Could you check a few things on this model? Use its own coordinates, in mm. A direction names the side the tool comes from. Give positions to 0.01 mm unless a question says otherwise; leave off trailing zeros. Write each loop counter-clockwise with the first axis right and the second up, starting at its lowest first coordinate (ties: lowest second). Pieces come first, ordered by that corner, then holes. Notation, with made-up numbers: (-39, -34.5) -> (-24, -34.5) arc R22 ccw to (-24, -13.5) -> close; hole circle Ø4 at (17, -36). An arc over 180 degrees is marked (long way). Write item = value, one per line. Start each with the question number.
```python
from build123d import *

# Parameters (mm, degrees)
BASE_BLOCK_DEPTH             = 80
UPRIGHT_NOTCHES_SKETCH_W     = 20
UPRIGHT_NOTCHES_SKETCH_H     = 10
UPRIGHT_TOP_NOTCHES_DEPTH    = 15
SADDLE_BORE_SKETCH_R         = 25
SADDLE_BORE_50_DEPTH         = 103.46950766
FRONT_SLOPE_CUT_DEPTH        = 111.742945599
FRONT_SLOT_SKETCH_W          = 5
FRONT_SLOT_SKETCH_H          = 40
FRONT_SLOT_40X5_DEPTH        = 11
FRONT_SLOT_UNDERCUT_SKETCH_W = 40
FRONT_SLOT_UNDERCUT_SKETCH_H = 8.064305279
FRONT_SLOT_UNDERCUT_DEPTH    = 11


with BuildPart() as part:
    # Base Profile Sketch → Base Block (new body)
    with BuildSketch(Plane.XY):
        Polygon((0, 0), (0, 50), (40, 50), (40, 20), (58, 20), (58, 0), align=None)
    extrude(amount=BASE_BLOCK_DEPTH)

    # Upright Notches Sketch → Upright Top Notches (cut)
    with BuildSketch(Plane(origin=(0, 50, 0), x_dir=(1, 0, 0), z_dir=(0, 1, 0))):
        with Locations((20, -13)):
            Rectangle(UPRIGHT_NOTCHES_SKETCH_W, UPRIGHT_NOTCHES_SKETCH_H)
        with Locations((20, -67)):
            Rectangle(UPRIGHT_NOTCHES_SKETCH_W, UPRIGHT_NOTCHES_SKETCH_H)
    extrude(amount=-UPRIGHT_TOP_NOTCHES_DEPTH, mode=Mode.SUBTRACT)

    # Saddle Bore Sketch → Saddle Bore Ø50 (cut, through all)
    with BuildSketch(Plane(origin=(40, 0, 0), x_dir=(0, 0, -1), z_dir=(1, 0, 0))):
        with Locations((-40, 50)):
            Circle(SADDLE_BORE_SKETCH_R)
    extrude(amount=-SADDLE_BORE_50_DEPTH, mode=Mode.SUBTRACT)

    # Front Slope Sketch → Front Slope Cut (cut, through all)
    with BuildSketch(Plane.XY.offset(80)):
        Polygon((50, 20), (58, 20), (58, 0), align=None)
    extrude(amount=-FRONT_SLOPE_CUT_DEPTH, mode=Mode.SUBTRACT)

    # Front Slot Sketch → Front Slot 40x5 (cut)
    with BuildSketch(Plane(origin=(0, 20, 0), x_dir=(1, 0, 0), z_dir=(0, 1, 0))):
        with Locations((47.5, -40)):
            Rectangle(FRONT_SLOT_SKETCH_W, FRONT_SLOT_SKETCH_H)
    extrude(amount=-FRONT_SLOT_40X5_DEPTH, mode=Mode.SUBTRACT)

    # Front Slot Undercut Sketch → Front Slot Undercut (cut)
    with BuildSketch(Plane(origin=(50, 20, 0), x_dir=(0, 0, -1), z_dir=(0.9284766908852593, 0.3713906763541041, 0))):
        with Locations((-40, -4.03215264)):
            Rectangle(FRONT_SLOT_UNDERCUT_SKETCH_W, FRONT_SLOT_UNDERCUT_SKETCH_H)
    extrude(amount=-FRONT_SLOT_UNDERCUT_DEPTH, mode=Mode.SUBTRACT)


solid = part.part
```
(1) On a 3-axis mill with a long thin cutter (end or side, diameter ignored), from which of +Z, -Z, +X, -X, +Y, -Y can I reach the whole of each face in a straight line? I mean faces 4 (the flat face through (30, 43, 68)), 5 (the flat face through (45, 19, 40)), 6 (the flat face through (41.263, 12.223, 40.28)). Say none if no direction works.
(2) Imagine slicing it at C-C (z = 69). Please give me the cut outline in (x, y), then the cut area to 3 significant figures.
(3) Imagine slicing it at D-D (y = 17). Please give me the cut outline in (x, z), then the cut area to 3 significant figures.
(4) Imagine slicing it at B-B (y = 28). Please give me the cut outline in (x, z), then the cut area to 3 significant figures.
(5) Imagine slicing it at A-A (x = 26.5). Please give me the cut outline in (y, z).
(6) If I drill on line 1 along Z through (x, y) = (46, 10); line 2 along X through (y, z) = (44.5, 69); line 3 along Y through (x, z) = (44, 48), over which ranges is the centre line in solid material (lowest first)? Write a range as from..to.
(7) I'm going to push flat-ended pins straight in: pin 1 (24 mm diameter, centred on y = 37, z = 54, fed in from +X); pin 2 (12 mm diameter, centred on x = 23, y = 44.5, fed in from -Z); pin 3 (5 mm diameter, centred on x = 40.5, z = 19.5, fed in from +Y); pin 4 (12 mm diameter, centred on x = 49.5, z = 27, fed in from +Y). Where does each tip first touch, or does it pass through?
(8) We'd pull the mould along Z, two halves only. Please class faces 1 (the flat face through (23, 25, 0)), 2 (the flat face through (40, 22, 39)), 3 (the flat face through (47, 9, 40)): released by +Z, released by -Z, zero draft, split by the parting line, or undercut.
Answers below:
q1.face_4 = +Y
q1.face_5 = +X, +Y
q1.face_6 = none
q2.outline = (0, 0) -> (58, 0) -> (50, 20) -> (40, 20) -> (40, 50) -> (30, 50) -> (30, 35) -> (10, 35) -> (10, 50) -> (0, 50) -> close
q2.area = 1,980 mm^2
q3.outline = (0, 0) -> (51.2, 0) -> (51.2, 20) -> (42.5, 20) -> (42.5, 60) -> (51.2, 60) -> (51.2, 80) -> (0, 80) -> close
q3.area = 3,750 mm^2
q4.outline = (0, 0) -> (40, 0) -> (40, 28.13) -> (0, 28.13) -> close; (0, 51.87) -> (40, 51.87) -> (40, 80) -> (0, 80) -> close
q4.area = 2,250 mm^2
q5.outline = (0, 0) -> (50, 0) -> (50, 8) -> (35, 8) -> (35, 18) -> (38.13, 18) arc R25 cw to (38.13, 62) -> (35, 62) -> (35, 72) -> (50, 72) -> (50, 80) -> (0, 80) -> close
q6.line_1 = 0..20, 60..80
q6.line_2 = 0..10, 30..40
q6.line_3 = 0..8.91, 17.6..20
q7.pin_1 = 40
q7.pin_2 = 0
q7.pin_3 = 40.08
q7.pin_4 = 20
q8.face_1 = released by -Z
q8.face_2 = zero draft
q8.face_3 = undercut
